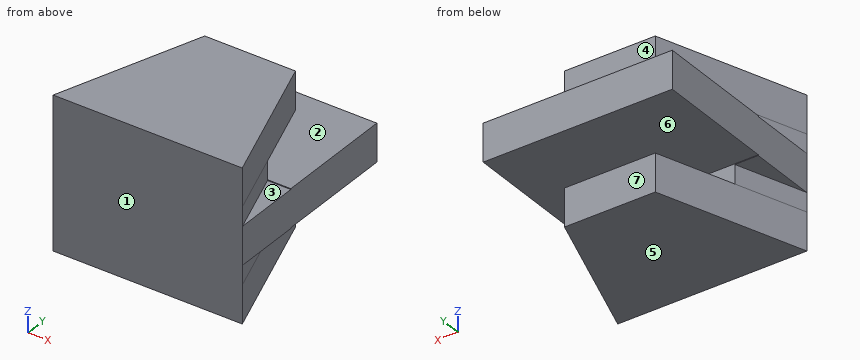
```python
from build123d import *

# Parameters (mm, degrees)
BASE_BLOCK_40MM_DEPTH       = 40
STEP_PROFILE_CUT_SKETCH_W   = 10
STEP_PROFILE_CUT_SKETCH_H   = 11.958807021
STEP_PROFILE_CUT_DEPTH      = 69.738635424
POCKET_24MM_X_10_DEEP_DEPTH = 10
POCKET_12MM_X_10_DEEP_DEPTH = 10
TRIANGULAR_CUT_A_5MM_DEPTH  = 5
TRIANGULAR_CUT_B_5MM_DEPTH  = 5
TRIANGULAR_CUT_C_5MM_DEPTH  = 5
TRIANGULAR_CUT_D_5MM_DEPTH  = 5


with BuildPart() as part:
    # Base Profile Sketch → Base Block 40mm (new body)
    with BuildSketch(Plane.XY):
        Polygon((12, 25), (-12, 25), (-25, 25), (-25, -25), (-12, 13), (12, 13), (25, -25), (25, 25), align=None)
        Polygon((12, 13), (25, -25), (-25, -25), (-12, 13), align=None)
    extrude(amount=BASE_BLOCK_40MM_DEPTH)

    # Step Profile Cut Sketch → Step Profile Cut (cut, through all)
    with BuildSketch(Plane(origin=(25, 0, 0), x_dir=(0, 0, -1), z_dir=(1, 0, 0))):
        Polygon((-25.21106926, -6.958807021), (-25.21106926, 25), (-30, 25), (-40, 25), (-40, 13.041192979), (-30, 13.041192979), (-30, -6.958807021), align=None)
        Polygon((-10, -6.958807021), (-10, 13.041192979), (-10, 25), (-15.21106926, 25), (-15.21106926, -6.958807021), align=None)
        with Locations((-5, 19.02059649)):
            Rectangle(STEP_PROFILE_CUT_SKETCH_W, STEP_PROFILE_CUT_SKETCH_H)
    extrude(amount=-STEP_PROFILE_CUT_DEPTH, mode=Mode.SUBTRACT)

    # Pocket 24mm Sketch → Pocket 24mm x 10 Deep (cut)
    with BuildSketch(Plane(origin=(0, 0, 0), x_dir=(-1, 0, 0), z_dir=(0, 0, -1))):
        Polygon((-12, 13.041192979), (12, 13.041192979), (25, -25), (25, 25), (-25, 25), (-25, -25), align=None)
    extrude(amount=-POCKET_24MM_X_10_DEEP_DEPTH, mode=Mode.SUBTRACT)

    # Pocket 12mm Sketch → Pocket 12mm x 10 Deep (cut)
    with BuildSketch(Plane.XY.offset(40)):
        Polygon((-25, -25), (-12, 13.041192979), (12, 13.041192979), (25, -25), (25, 25), (-25, 25), align=None)
    extrude(amount=-POCKET_12MM_X_10_DEEP_DEPTH, mode=Mode.SUBTRACT)

    # Triangular Cut A Sketch → Triangular Cut A 5mm (cut)
    with BuildSketch(Plane.XY.offset(30)):
        Polygon((-25, -25), (-25, -6.958807021), (-18.834696276, -6.958807021), align=None)
    extrude(amount=-TRIANGULAR_CUT_A_5MM_DEPTH, mode=Mode.SUBTRACT)

    # Triangular Cut B Sketch → Triangular Cut B 5mm (cut)
    with BuildSketch(Plane(origin=(0, 0, 10), x_dir=(-1, 0, 0), z_dir=(0, 0, -1))):
        Polygon((25, -25), (25, -6.958807021), (18.834696276, -6.958807021), align=None)
    extrude(amount=-TRIANGULAR_CUT_B_5MM_DEPTH, mode=Mode.SUBTRACT)

    # Triangular Cut C Sketch → Triangular Cut C 5mm (cut)
    with BuildSketch(Plane(origin=(0, 0, 10), x_dir=(-1, 0, 0), z_dir=(0, 0, -1))):
        Polygon((-25, -25), (-18.834696276, -6.958807021), (-25, -6.958807021), align=None)
    extrude(amount=-TRIANGULAR_CUT_C_5MM_DEPTH, mode=Mode.SUBTRACT)

    # Triangular Cut D Sketch → Triangular Cut D 5mm (cut)
    with BuildSketch(Plane.XY.offset(30)):
        Polygon((25, -25), (25, -6.958807021), (18.834696276, -6.958807021), align=None)
    extrude(amount=-TRIANGULAR_CUT_D_5MM_DEPTH, mode=Mode.SUBTRACT)


solid = part.part
```
Model file for the job. Use its own axes, mm. Face numbers are marked on the shaded views. A direction names the side the tool comes from. Coordinates: 2 decimals unless noted, no trailing zeros. Order: outer loops, then holes, each group sorted by start corner. A loop starts at its lowest first (then second) coordinate and runs counter-clockwise, first axis right, second up. Notation, with made-up numbers: (0, 88) - (19, 88) arc R25 cw to (19, 106) - close; hole circle Ø1 at (-11, 6.25). An arc over 180 degrees is marked (long way). Return JSON: item names as keys, results as strings. Group by question number.
1) Saw through at D-D, the plane z = 27.5. Write the cut outline in (x, y).
2) Probe line 1 (Z direction, x = -3, y = -3); line 2 (Z direction, x = 2, y = 13.5); line 3 (Y direction, x = -5.5, z = 2.5). List the from-to ranges inside material, lowest first. Write a range as from..to.
3) Saw through at C-C, the plane y = -19.5. Write the cut outline in (x, z), plus the area to 3 significant figures.
4) Saw through at A-A, the plane y = -4. Write the cut outline in (x, z), plus the area to 3 significant figures.
5) Tool access for the marked faces 1, 2, 3 and 4: list every direction of +Z, -Z, +X, -X, +Y, -Y with a clear straight run to the whole face (end or side of a thin tool).
6) Saw through at B-B, the plane x = 8.5. Write the cut outline in (y, z), plus the area to 3 significant figures.
7) Flat gauge pins, fed straight in: P1, Ø11, axis at x = -1.5, z = 34.5, coming from the +Y side; P2, Ø3, axis at x = -6, y = 17, coming from the +Z side; P3, Ø1.8, axis at x = -22, y = -11.5, coming from the +Z side. Where does each tip first touch, or does it go through?
8) Mould opens along Z. For the marked faces 5, 6 and 7 say: released by +Z, released by -Z, zero draft, split by the parting line, or undercut.
Values found:
{
 "1": {"outline": "(-25, -25) - (25, -25) - (18.83, -6.96) - (-18.83, -6.96) - close"},
 "2": {"line 1": "z = 0..10, 15.21..25.21, 30..40", "line 2": "z = 15.21..25.21", "line 3": "y = -25..13.04"},
 "3": {"outline": "(-25, 15) - (-23.12, 15) - (-23.12, 0) - (23.12, 0) - (23.12, 15) - (25, 15) - (25, 25) - (23.12, 25) - (23.12, 40) - (-23.12, 40) - (-23.12, 25) - (-25, 25) - close", "area": "1,890 mm²"},
 "4": {"outline": "(-25, 15.21) - (25, 15.21) - (25, 25.21) - (-25, 25.21) - close; (-17.82, 0) - (17.82, 0) - (17.82, 10) - (-17.82, 10) - close; (-17.82, 30) - (17.82, 30) - (17.82, 40) - (-17.82, 40) - close", "area": "1,210 mm²"},
 "5": {"face 1": "+Z, -Z, +X, -X, -Y", "face 2": "+X, -X, +Y", "face 3": "+Z, +X", "face 4": "+Z, +X, -X, +Y"},
 "6": {"outline": "(-25, 0) - (13.04, 0) - (13.04, 10) - (-6.96, 10) - (-6.96, 15.21) - (25, 15.21) - (25, 25.21) - (-6.96, 25.21) - (-6.96, 30) - (13.04, 30) - (13.04, 40) - (-25, 40) - close", "area": "1,440 mm²"},
 "7": {"P1": "stops at y = 13.04", "P2": "stops at z = 25.21", "P3": "stops at z = 25"},
 "8": {"face 5": "released by -Z", "face 6": "undercut", "face 7": "zero draft"}
}
